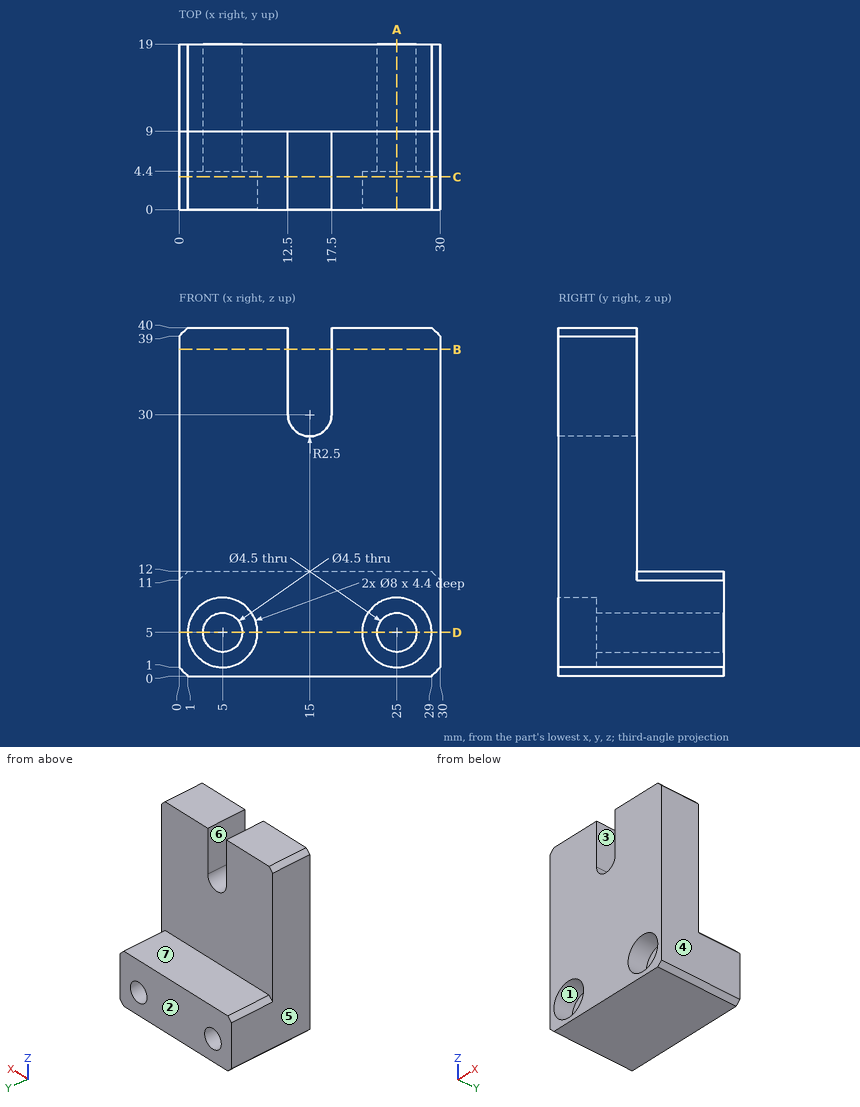
Here's the drawing with two shaded views (mm, measured from the low corner). I have some questions. A direction names the side the tool comes from. Coordinates: 2 decimals unless noted, no trailing zeros. Loops run counter-clockwise (first coordinate to the right, second up) from the corner with the lowest first, then second, coordinate; pieces in that order, holes last. Notation, with made-up numbers: M 82,35 L 99,35 A22 cw 99,47 Z; hole C 59,61.25 d4. An arc over 180 degrees is marked long. Return JSON: item names as keys, results as strings. Group by question number.
Item 1: If I drill on L1, parallel to X at y = 14, z = 5; L2, parallel to X at y = 2.75, z = 38; L3, parallel to Z at x = 5, y = 8, over which ranges is the centre line in solid material (lowest first)? Write a range as from..to.
Item 2: Imagine slicing it at A-A (x = 25). Please give me the cut outline in (y, z), and give its area (3 significant figures).
Item 3: On a 3-axis mill with a long thin cutter (end or side, diameter ignored), from which of +Z, -Z, +X, -X, +Y, -Y can I reach the whole of each face in a straight line? I mean the marked faces 1, 2 and 3. Say none if no direction works.
Item 4: I'm going to push flat-ended pins straight in: pin 1 Ø8 at (x, z) = (13, 25.5) entering from +Y; pin 2 Ø3.5 at (x, z) = (25, 5) entering from +Y; pin 3 Ø2.5 at (x, z) = (23.5, 6.5) entering from -Y. Where does each tip first touch, or does it pass through?
Item 5: Imagine slicing it at C-C (y = 3.75). Please give me the cut outline in (x, z).
Item 6: Imagine slicing it at D-D (z = 5). Please give me the cut outline in (x, y).
Item 7: Imagine slicing it at B-B (z = 37.5). Please give me the cut outline in (x, y).
Item 8: Thinking about a two-plate mould opening in X: for the marked faces 4, 5, 6 and 7, which applies, released by +X, released by -X, zero draft, split by the parting line, or undercut?
Verdict:
{
 "1": {"L1": "x = 0..2.75, 7.25..22.75, 27.25..30", "L2": "x = 0..12.5, 17.5..30", "L3": "z = 0..2.75, 7.25..40"},
 "2": {"outline": "M 0,0 L 19,0 L 19,2.75 L 4.4,2.75 L 4.4,1 L 0,1 Z; M 0,9 L 4.4,9 L 4.4,7.25 L 19,7.25 L 19,12 L 9,12 L 9,40 L 0,40 Z", "area": "379 mm^2"},
 "3": {"face 1": "-Y", "face 2": "+Z, -Z, +X, -X, +Y", "face 3": "+Z, +Y, -Y"},
 "4": {"pin 1": "stops at y = 9", "pin 2": "passes through", "pin 3": "stops at y = 4.4"},
 "5": {"outline": "M 0,1 L 1,0 L 29,0 L 30,1 L 30,39 L 29,40 L 17.5,40 L 17.5,30 A2.5 cw 12.5,30 L 12.5,40 L 1,40 L 0,39 Z; hole C 5,5 d8; hole C 25,5 d8"},
 "6": {"outline": "M 0,0 L 1,0 L 1,4.4 L 2.75,4.4 L 2.75,19 L 0,19 Z; M 7.25,4.4 L 9,4.4 L 9,0 L 21,0 L 21,4.4 L 22.75,4.4 L 22.75,19 L 7.25,19 Z; M 27.25,4.4 L 29,4.4 L 29,0 L 30,0 L 30,19 L 27.25,19 Z"},
 "7": {"outline": "M 0,0 L 12.5,0 L 12.5,9 L 0,9 Z; M 17.5,0 L 30,0 L 30,9 L 17.5,9 Z"},
 "8": {"face 4": "released by +X", "face 5": "released by -X", "face 6": "undercut", "face 7": "zero draft"}
}
